Could you check a few things on this drawing? It's one solid part, dimensions in mm from its lowest x, y, z. A direction names the side the tool comes from. Give positions to 0.01 mm unless a question says otherwise; leave off trailing zeros. Order: outer loops, then holes, each group sorted by start corner. A loop starts at its lowest first (then second) coordinate and runs counter-clockwise, first axis right, second up. Notation, with made-up numbers: M 83,60 L 133,60 A24 cw 133,80 Z; hole C 39.25,-35.75 d2. An arc over 180 degrees is marked long. Use one line per item in the form item = value.
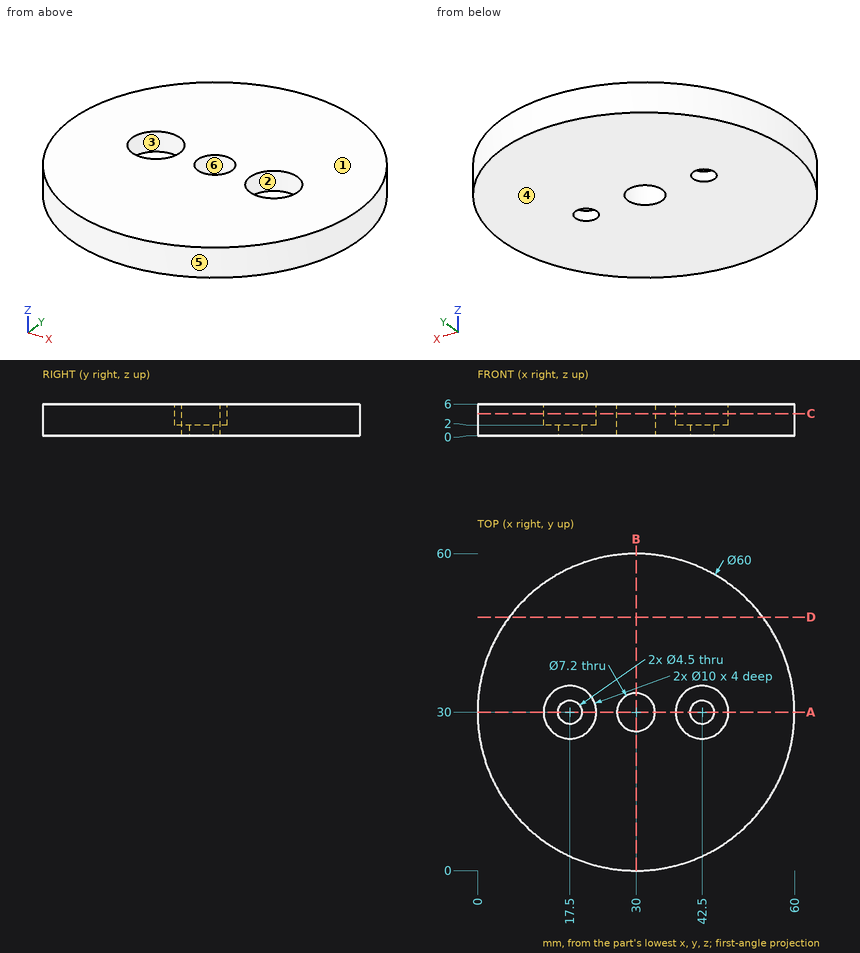
Q1. I need wall thicknesses on L1, parallel to X at y = 31, z = 2.6; L2, parallel to Y at x = 33, z = 3.85; L3, parallel to Y at x = 46.5, z = 4.85. Which ranges of each line are inside material? Lowest first, please.
Found:
L1 = 0.02 to 12.6, 22.4 to 26.54, 33.46 to 37.6, 47.4 to 59.98
L2 = 0.15 to 28.01, 31.99 to 59.85
L3 = 4.95 to 27, 33 to 55.05
Q2. I want a section at D-D on y = 48. Write out the boundary of the cut face in (x, z).
Found:
outline = M 6,0 L 54,0 L 54,6 L 6,6 Z
Q3. I want a section at A-A on y = 30. Write out the boundary of the cut face in (x, z), then the cut area to 3 significant figures.
Found:
outline = M 0,0 L 15.25,0 L 15.25,2 L 12.5,2 L 12.5,6 L 0,6 Z; M 19.75,0 L 26.4,0 L 26.4,6 L 22.5,6 L 22.5,2 L 19.75,2 Z; M 33.6,0 L 40.25,0 L 40.25,2 L 37.5,2 L 37.5,6 L 33.6,6 Z; M 44.75,0 L 60,0 L 60,6 L 47.5,6 L 47.5,2 L 44.75,2 Z
area = 219 mm²
Q4. I want a section at B-B on x = 30. Write out the boundary of the cut face in (y, z), then the cut area to 3 significant figures.
Found:
outline = M 0,0 L 26.4,0 L 26.4,6 L 0,6 Z; M 33.6,0 L 60,0 L 60,6 L 33.6,6 Z
area = 317 mm²
Q5. Thinking about a two-plate mould opening in X: for the marked faces 3, 4, 5 and 6, which applies, +X half, -X half, draft (parallel to the pull), parting line (faces both ways), or undercut?
Found:
face_3 = undercut
face_4 = draft
face_5 = parting line
face_6 = undercut
Q6. I'm going to push flat-ended pins straight in: pin 1 Ø3 at (y, z) = (26.5, 1) entering from -X; pin 2 Ø3 at (y, z) = (19, 2.5) entering from +X; pin 3 Ø5 at (x, y) = (42.5, 28.5) entering from +Z; pin 4 Ø6 at (x, y) = (30, 30) entering from +Z. Where does each tip first touch, or does it pass through?
Found:
pin_1 = 0.07
pin_2 = 58.46
pin_3 = 2
pin_4 = through
Q7. On a 3-axis mill with a long thin cutter (end or side, diameter ignored), from which of +Z, -Z, +X, -X, +Y, -Y can I reach the whole of each face in a straight line? I mean the marked faces 1 and 2. Say none if no direction works.
Found:
face_1 = +Z, +X, -X, +Y, -Y
face_2 = +Z
Q8. I want a section at C-C on z = 4.2. Write out the boundary of the cut face in (x, y).
Found:
outline = C 30,30 d60; hole C 17.5,30 d10; hole C 30,30 d7.2; hole C 42.5,30 d10
